Work out the finished part from the listing and answer in its coordinate system (mm). A direction names the side the tool comes from. Round coordinates to 2 decimals unless told otherwise and drop trailing zeros. Loops run counter-clockwise (first coordinate to the right, second up) from the corner with the lowest first, then second, coordinate; pieces in that order, holes last.
```python
from build123d import *

# Parameters (mm, degrees)
BASE_PLATE_SKETCH_R   = 4
BASE_PLATE_DEPTH      = 11
GUIDE_BLOCK_DEPTH     = 26
CENTRE_SLOT_CUT_DEPTH = 26


with BuildPart() as part:
    # Base Plate Sketch → Base Plate (new body)
    with BuildSketch(Plane.XY):
        with BuildLine():
            Line((-54, 27), (54, 27))
            Line((54, 27), (54, -17))
            ThreePointArc((54, -17), (51.071067812, -24.071067812), (44, -27))
            Line((44, -27), (-44, -27))
            ThreePointArc((-44, -27), (-51.071067812, -24.071067812), (-54, -17))
            Line((-54, -17), (-54, 27))
        make_face()
        with Locations((-45.682264333, 17)):
            Circle(BASE_PLATE_SKETCH_R, mode=Mode.SUBTRACT)
        with Locations((-45.682264333, -8)):
            Circle(BASE_PLATE_SKETCH_R, mode=Mode.SUBTRACT)
        with Locations(Location((45.682264333, -8, 0), (0, 0, 180))):
            Circle(BASE_PLATE_SKETCH_R, mode=Mode.SUBTRACT)
        with Locations(Location((45.682264333, 17, 0), (0, 0, 180))):
            Circle(BASE_PLATE_SKETCH_R, mode=Mode.SUBTRACT)
    extrude(amount=BASE_PLATE_DEPTH)

    # Guide Block Profile → Guide Block (add, symmetric)
    with BuildSketch(Plane(origin=(0, 0, 0), x_dir=(0, 0, -1), z_dir=(1, 0, 0))):
        with BuildLine():
            Line((-11, 21), (-23, 21))
            Line((-23, 21), (-23, 15))
            Line((-23, 15), (-32, 15))
            ThreePointArc((-32, 15), (-26.8587637, -8.67938185), (-11, -27))
            Line((-11, -27), (-11, 21))
        make_face()
    extrude(amount=GUIDE_BLOCK_DEPTH, both=True)

    # Centre Slot Sketch → Centre Slot Cut (cut, symmetric)
    with BuildSketch(Plane(origin=(0, 0, 0), x_dir=(1, 0, 0), z_dir=(0, 1, 0))):
        Polygon((-9, -17), (-23.387504735, -43.976571377), (23.387504735, -43.976571377), (9, -17), align=None)
    extrude(amount=CENTRE_SLOT_CUT_DEPTH, both=True, mode=Mode.SUBTRACT)


solid = part.part
```
1. Find section C-C (x = -18.5). Write down the section's boundary in (y, z).
Answer key:
outline: (-27, 0) - (27, 0) - (27, 11) - (21, 11) - (21, 23) - (15, 23) - (15, 32) arc R49 ccw to (-27, 11) - close
2. Determine the mould class of faces 1 (the face through (54, 5, 5)), 2 (the face through (1, -27, 5)), 3 (the face through (49.68, 16.82, 5.42)) for opening direction Y: +Y half, -Y half, draft (parallel to the pull), parting line (faces both ways), or undercut.
Answer key:
face 1: draft
face 2: -Y half
face 3: undercut
3. Find section B-B (y = 17). Write down the section's boundary in (x, z).
Answer key:
outline: (-54, 0) - (-49.68, 0) - (-49.68, 11) - (-54, 11) - close; (-41.68, 0) - (41.68, 0) - (41.68, 11) - (26, 11) - (26, 23) - (12.2, 23) - (9, 17) - (-9, 17) - (-12.2, 23) - (-26, 23) - (-26, 11) - (-41.68, 11) - close; (49.68, 0) - (54, 0) - (54, 11) - (49.68, 11) - close
4. Which of the six approach directions +Z, -Z, +X, -X, +Y, -Y give full straight-line access (tool end or side, diameter ignored) to faces 4 (the face through (26, 3, 19)), 5 (the face through (-54, 5, 5)), 6 (the face through (-26, 3, 19)), 7 (the face through (12.2, 4.5, 23)), 8 (the face through (0, 21, 16))?
Answer key:
face 4: +Z, +X, +Y, -Y
face 5: +Z, -Z, -X, +Y, -Y
face 6: +Z, -X, +Y, -Y
face 7: +Z, +Y, -Y
face 8: +Z, +X, -X, +Y
5. Find section D-D (z = 25). Write down the section's boundary in (x, y), then the cut area to 3 significant figures.
Answer key:
outline: (-26, -12.06) - (-13.27, -12.06) - (-13.27, 15) - (-26, 15) - close; (13.27, -12.06) - (26, -12.06) - (26, 15) - (13.27, 15) - close
area: 689 mm2
6. Consider probe 1 along X at (y, z) = (16.5, 3); probe 2 along Z at (x, y) = (-29.5, -7); probe 3 along X at (y, z) = (6.5, 19.5). Determine where each line is inside the solid, lowest interval first.
Answer key:
probe 1: x = -54 to -49.65, -41.71 to 41.71, 49.65 to 54
probe 2: z = 0 to 11
probe 3: x = -26 to -10.33, 10.33 to 26
7. Find section A-A (z = 6). Write down the section's boundary in (x, y).
Answer key:
outline: (-54, -17) arc R10 ccw to (-44, -27) - (44, -27) arc R10 ccw to (54, -17) - (54, 27) - (-54, 27) - close; hole circle Ø8 at (-45.68, -8); hole circle Ø8 at (-45.68, 17); hole circle Ø8 at (45.68, -8); hole circle Ø8 at (45.68, 17)
8. Given pin 1 (1 mm diameter, centred on y = 9, z = 23.5, fed in from +X); pin 2 (6.5 mm diameter, centred on x = -16.5, y = 18, fed in from +Z); pin 3 (4.5 mm diameter, centred on x = -21.5, z = 26, fed in from +Y), each flat-ended and moving along its own axis, determine where each tip first touches the part or whether it passes through.
Answer key:
pin 1: stops at x = 26
pin 2: stops at z = 32.01
pin 3: stops at y = 15
